Read the model definition and answer for the solid it produces. Units are mm, in the model's axes. A direction names the side the tool comes from. Coordinates: 2 decimals unless noted, no trailing zeros. Order: outer loops, then holes, each group sorted by start corner. A loop starts at its lowest first (then second) coordinate and runs counter-clockwise, first axis right, second up. Notation, with made-up numbers: (37.5, 7.25) - (59.5, 7.25) arc R8 cw to (59.5, 19.25) - close; hole circle Ø7 at (35.25, -9). An arc over 180 degrees is marked (long way). Use one line per item in the form item = value.
```python
from build123d import *

# Parameters (mm, degrees)
SKETCH1_W           = 50
SKETCH1_H           = 53.7
BOSS_EXTRUDE1_DEPTH = 30
SHELL1_T            = -3
CUT_EXTRUDE1_DEPTH  = 66
FILLET1_R           = 3
FILLET2_R           = 1


with BuildPart() as part:
    # Sketch1 → Boss-Extrude1 (new body)
    with BuildSketch(Plane.XY):
        Rectangle(SKETCH1_W, SKETCH1_H)
    extrude(amount=BOSS_EXTRUDE1_DEPTH)

    # Shell1
    shell1_openings = [part.faces().sort_by_distance(p)[0] for p in [
        (0, -26.85, 15),
        (0, 26.85, 15),
    ]]
    offset(amount=SHELL1_T, openings=shell1_openings, kind=Kind.INTERSECTION)

    # Sketch2 → Cut-Extrude1 (cut)
    with BuildSketch(Plane(origin=(25, 0, 0), x_dir=(0, 0, -1), z_dir=(1, 0, 0))):
        with BuildLine():
            Line((-11.212154068, 15.401262658), (13.536583273, 40.15))
            Line((13.536583273, 40.15), (-14.747687974, 68.434271247))
            Line((-14.747687974, 68.434271247), (-43.031959221, 40.15))
            Line((-43.031959221, 40.15), (-18.28322188, 15.401262658))
            ThreePointArc((-18.28322188, 15.401262658), (-14.747687974, 13.936796564), (-11.212154068, 15.401262658))
        make_face()
    extrude(amount=-CUT_EXTRUDE1_DEPTH, mode=Mode.SUBTRACT)

    # Fillet1
    fillet1_edges = [part.edges().sort_by_distance(p)[0] for p in [
        (-25, -0.118291637, 0),
        (25, -0.118291637, 0),
        (-25, 0, 30),
        (25, 0, 30),
    ]]
    fillet(fillet1_edges, radius=FILLET1_R)

    # Fillet2
    fillet2_edges = [part.edges().sort_by_distance(p)[0] for p in [
        (22, -1.618291637, 3),
        (22, -1.365979611, 27),
        (-22, -1.618291637, 3),
        (-22, -1.365979611, 27),
    ]]
    fillet(fillet2_edges, radius=FILLET2_R)


solid = part.part
```
(1) Which of the six approach directions +Z, -Z, +X, -X, +Y, -Y give full straight-line access (tool end or side, diameter ignored) to faces 4 (the flat face through (0, -1, 27)), 5 (the flat face through (1.969, 23.888, 2.725)), 6 (the cylindrical face through (-24.14, 0.38, 29.1))?
Answer list:
face_4 = +Y, -Y
face_5 = +X, -X, +Y
face_6 = +Z, -X, +Y, -Y
(2) Section A-A, the plane x = -11.5 is taken. Write down the section's boundary in (y, z), then the cut area to 3 significant figures.
Answer list:
outline = (-26.85, 0) - (26.61, 0) - (23.61, 3) - (-26.85, 3) - close; (-26.85, 27) - (24.12, 27) - (26.85, 29.73) - (26.85, 30) - (-26.85, 30) - close
area = 313 mm2
(3) Section C-C, the plane z = 9 is taken. Write down the section's boundary in (x, y).
Answer list:
outline = (-25, -26.85) - (-22, -26.85) - (-22, 17.61) - (-25, 17.61) - close; (22, -26.85) - (25, -26.85) - (25, 17.61) - (22, 17.61) - close
(4) Section D-D, the plane z = 19.25 is taken. Write down the section's boundary in (x, y).
Answer list:
outline = (-25, -26.85) - (-22, -26.85) - (-22, 16.37) - (-25, 16.37) - close; (22, -26.85) - (25, -26.85) - (25, 16.37) - (22, 16.37) - close
(5) Section B-B, the plane y = -1.5 is taken. Write down the section's boundary in (x, z).
Answer list:
outline = (-25, 3) arc R3 ccw to (-22, 0) - (22, 0) arc R3 ccw to (25, 3) - (25, 27) arc R3 ccw to (22, 30) - (-22, 30) arc R3 ccw to (-25, 27) - close; hole (-22, 4) arc R1 ccw to (-21, 3) - (21, 3) arc R1 ccw to (22, 4) - (22, 26) arc R1 ccw to (21, 27) - (-21, 27) arc R1 ccw to (-22, 26) - close
(6) Straight lines are drawn through the part: L1, parallel to X at y = 7, z = 23.5; L2, parallel to Z at x = 0, y = 16; L3, parallel to Z at x = -22.5, y = 22.5. For each, find the intervals that lie inside material, in ascending order.
Answer list:
L1 = -25 to -22, 22 to 25
L2 = 0 to 3, 27 to 30
L3 = 0.04 to 4.11, 25.38 to 29.96
(7) The mould has two halves that part along X. Classify faces 1 (the flat face through (22, -2, 15)), 2 (the flat face through (-25, -7, 15)), 3 (the cylindrical face through (24.1, 0.26, 0.86)): +X half, -X half, draft (parallel to the pull), parting line (faces both ways), or undercut.
Answer list:
face_1 = undercut
face_2 = -X half
face_3 = +X half
